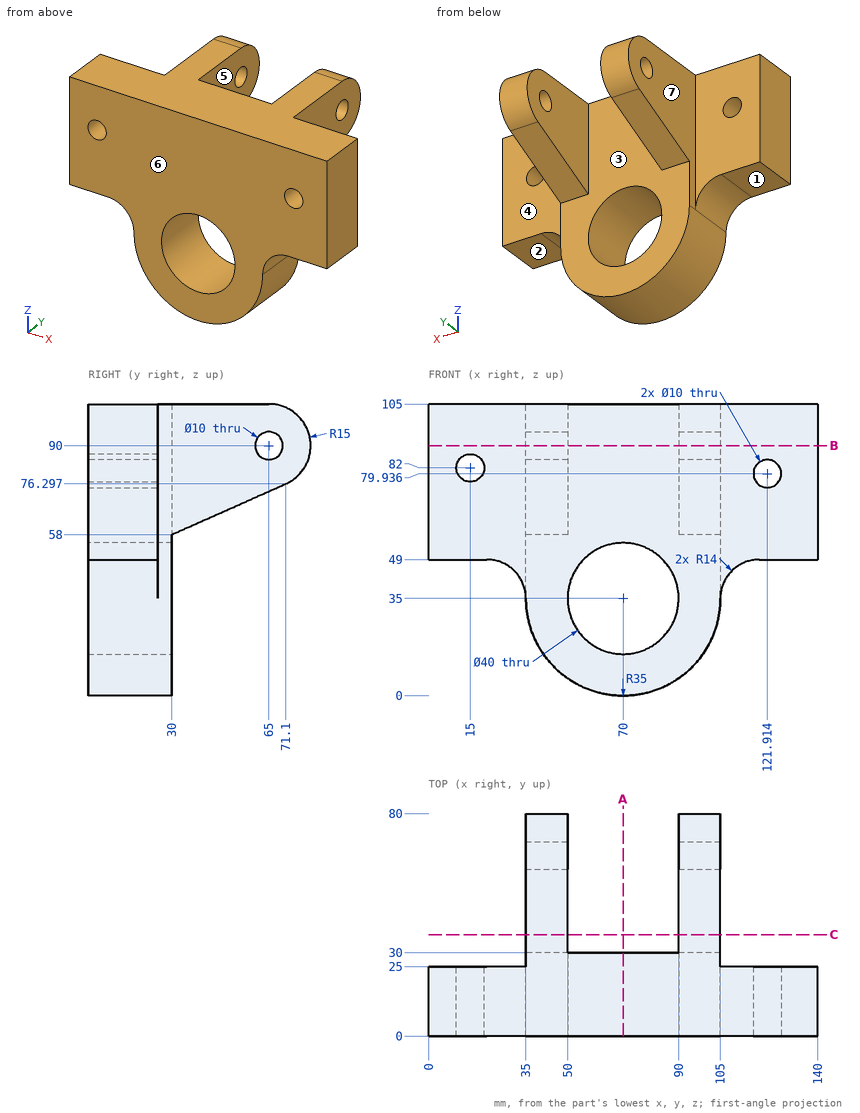
Print and shaded views of the part. All mm, measured from the part's lowest x, y and z. A direction names the side the tool comes from. Coordinates: 2 decimals unless noted, no trailing zeros. Write each loop counter-clockwise with the first axis right and the second up, starting at its lowest first coordinate (ties: lowest second). Pieces come first, ordered by that corner, then holes.
(1) Flat gauge pins, fed straight in: pin 1 (1.5 mm diameter, centred on x = 117, z = 71.5, fed in from +Y); pin 2 (23.5 mm diameter, centred on y = 51.5, z = 93, fed in from -X); pin 3 (1 mm diameter, centred on x = 84.5, z = 48.5, fed in from +Y). Where does each tip first touch, or does it go through?
(2) Cut at A-A, the plane x = 70. List the corners of the cut face in (y, z).
(3) 3-axis set-ups, long thin cutter, end or side, ignore diameter. For the marked faces 1, 2, 3 and 4: which of +Z, -Z, +X, -X, +Y, -Y reach the whole face in a straight line?
(4) Cut at C-C, the plane y = 36.5. List the corners of the cut face in (x, z).
(5) Drill centre lines: probe 1 along X at (y, z) = (48, 68); probe 2 along Y at (x, z) = (95, 90); probe 3 along X at (y, z) = (15, 82). Where is each one in solid material? Low to high.
(6) Two-plate mould, pull along X, no slides. Class the marked faces 5, 6 and 7: +X half, -X half, draft (parallel to the pull), parting line (faces both ways), or undercut.
(7) Cut at B-B, the plane z = 90. List the corners of the cut face in (x, y).
Geometry says:
1. pin 1: stops at y = 25
1. pin 2: stops at x = 35
1. pin 3: stops at y = 30
2. outline: (0, 0) - (30, 0) - (30, 15) - (0, 15) - close; (0, 55) - (30, 55) - (30, 105) - (0, 105) - close
3. face 1: -Z, -X, +Y, -Y
3. face 2: -Z, +X, +Y, -Y
3. face 3: -Z, +Y
3. face 4: +Z, -Z, +X, +Y
4. outline: (35, 60.89) - (50, 60.89) - (50, 105) - (35, 105) - close; (90, 60.89) - (105, 60.89) - (105, 105) - (90, 105) - close
5. probe 1: x = 35 to 50, 90 to 105
5. probe 2: y = 0 to 60, 70 to 80
5. probe 3: x = 0 to 10, 20 to 117.36, 126.47 to 140
6. face 5: undercut
6. face 6: draft
6. face 7: -X half
7. outline: (0, 0) - (140, 0) - (140, 25) - (105, 25) - (105, 60) - (90, 60) - (90, 30) - (50, 30) - (50, 60) - (35, 60) - (35, 25) - (0, 25) - close; (35, 70) - (50, 70) - (50, 80) - (35, 80) - close; (90, 70) - (105, 70) - (105, 80) - (90, 80) - close
